Source: CAD feature listing. Evaluate the final solid. Frame: model axes, mm. A direction names the side the tool comes from. Give positions to 0.01 mm unless a question says otherwise; leave off trailing zeros. Loops run counter-clockwise (first coordinate to the right, second up) from the corner with the lowest first, then second, coordinate; pieces in that order, holes last. Notation, with made-up numbers: M -7.5,58.25 L 37.5,58.25 A19 cw 37.5,88.25 Z; hole C 70,10.25 d7. An arc over 180 degrees is marked long. Answer in a Markdown table with one row per item.
```python
from build123d import *

# Parameters (mm, degrees)
SKETCH4_OUTSIDE_W  = 15.98
SKETCH4_OUTSIDE_H  = 15.98
CUT_EXTRUDE2_DEPTH = 3
CHAMFER1_SIZE      = 0.5
CHAMFER2_SIZE      = 0.2


with BuildPart() as part:
    # Sketch2 → Revolve1 (revolve)
    with BuildSketch(Plane.XY, mode=Mode.PRIVATE) as revolve1_sk:
        Polygon((0, 0), (2.5, 0), (2.5, 6), (5, 6), (5, 7), (4, 7), (4, 14), (0, 14), align=None)
    revolve(revolve1_sk.sketch.rotate(Axis((0, 0, 0), (0, 1, 0)), 90), axis=Axis((0, 0, 0), (0, 1, 0)))

    # Sketch4 outside → Cut-Extrude2 (cut)
    with BuildSketch(Plane(origin=(0, 14, 0), x_dir=(1, 0, 0), z_dir=(0, 1, 0))):
        Rectangle(SKETCH4_OUTSIDE_W, SKETCH4_OUTSIDE_H)
        Polygon((1.732050808, 3), (-1.732050808, 3), (-3.464101615, 0), (-1.732050808, -3), (1.732050808, -3), (3.464101615, 0), align=None, mode=Mode.SUBTRACT)
    extrude(amount=-CUT_EXTRUDE2_DEPTH, mode=Mode.SUBTRACT)

    # Chamfer1
    chamfer1_edges = [part.edges().sort_by_distance(p)[0] for p in [
        (2.598076211, 14, -1.5),
        (2.598076211, 14, 1.5),
        (0, 14, 3),
        (-2.598076211, 14, 1.5),
        (-2.598076211, 14, -1.5),
        (0, 14, -3),
        (0, 0, 2.5),
    ]]
    chamfer(chamfer1_edges, length=CHAMFER1_SIZE)

    # Chamfer2
    chamfer2_edges = [part.edges().sort_by_distance(p)[0] for p in [
        (0, 11, 4),
        (0, 7, 5),
        (0, 6, 5),
    ]]
    chamfer(chamfer2_edges, length=CHAMFER2_SIZE)


solid = part.part
```
1) Pin query (flat end, axial travel): pin 1 Ø4 at (y, z) = (5.5, 1) entering from +X; pin 2 Ø0.8 at (x, y) = (-0.5, 12) entering from +Z; pin 3 Ø0.8 at (x, y) = (-0.5, 12.5) entering from -Z; pin 4 Ø4 at (x, y) = (-3, 12.5) entering from -Z. Return the tip coordinate at first contact, or that it passes through.
Reply:
| item | result |
|---|---|
| pin 1 | stops at x = 5 |
| pin 2 | stops at z = 3 |
| pin 3 | stops at z = -3 |
| pin 4 | stops at z = -3.49 |
2) Section B-B, the plane y = 4.25. Return loops of the section in (x, z), then the cut area to 3 significant figures.
Reply:
| item | result |
|---|---|
| outline | C 0,0 d5 |
| area | 19.6 mm² |
3) Section A-A, the plane x = 0. Return loops of the section in (y, z), then the cut area to 3 significant figures.
Reply:
| item | result |
|---|---|
| outline | M 0,-2 L 0.5,-2.5 L 6,-2.5 L 6,-4.8 L 6.2,-5 L 6.8,-5 L 7,-4.8 L 7,-4 L 10.8,-4 L 11,-3.8 L 11,-3 L 13.5,-3 L 14,-2.5 L 14,2.5 L 13.5,3 L 11,3 L 11,3.8 L 10.8,4 L 7,4 L 7,4.8 L 6.8,5 L 6.2,5 L 6,4.8 L 6,2.5 L 0.5,2.5 L 0,2 Z |
| area | 89.4 mm² |
4) Material intervals for L1, parallel to Y at x = 4.25, z = 2; L2, parallel to Y at x = 2.25, z = -3; L3, parallel to Z at x = 1, y = 12.75, sorted ascending.
Reply:
| item | result |
|---|---|
| L1 | y = 6 to 7 |
| L2 | y = 6 to 11 |
| L3 | z = -3 to 3 |
5) Set-up query: faces 1 (the flat face through (-2.6, 12.3, -1.5)), 2 (the flat face through (-2.6, 12.3, 1.5)), 3 (the flat face through (-4, 7, 2)), 4 (the flat face through (2.6, 12.3, -1.5)). Return all of +Z, -Z, +X, -X, +Y, -Y with unobstructed straight access to the full face (end or side cutting, diameter ignored); none if empty.
Reply:
| item | result |
|---|---|
| face 1 | -Z, -X, +Y |
| face 2 | +Z, -X, +Y |
| face 3 | +Y |
| face 4 | -Z, +X, +Y |
